Here's how the part is built. I have some questions about the finished solid (model axes, mm). A direction names the side the tool comes from. Coordinates: 2 decimals unless noted, no trailing zeros. Loops run counter-clockwise (first coordinate to the right, second up) from the corner with the lowest first, then second, coordinate; pieces in that order, holes last. Notation, with made-up numbers: (16.5, -27.75) -> (62.5, -27.75) arc R18 ccw to (62.5, -20.75) -> close; hole circle Ø4 at (24, 85.25). An arc over 180 degrees is marked (long way). Answer as a JSON object with one key per item and string values. Group by question number.
Q1. I want a section at A-A on y = 43. Write out the boundary of the cut face in (x, z).
Q2. I need wall thicknesses on line 1 (Z direction, x = 0, y = 80); line 2 (Z direction, x = 0, y = -6.5); line 3 (X direction, y = 84.5, z = -7.5). Which ranges of each line are inside material? Lowest first, please.
Q3. On a 3-axis mill with a long thin cutter (end or side, diameter ignored), from which of +Z, -Z, +X, -X, +Y, -Y can I reach the whole of each face in a straight line? I mean faces 1 (the cylindrical face through (-6.586, 73.801, -10.329)), 2 (the flat face through (7.3, 92.053, -10.1)), 3 (the cylindrical face through (2.285, -11.807, -3.584)), 4 (the flat face through (-14, 84, 0)), 5 (the flat face through (14, 84, 0)). Say none if no direction works.
Q4. I'm going to push flat-ended pins straight in: pin 1 (6 mm diameter, centred on x = -16.5, y = 47, fed in from +Z); pin 2 (12 mm diameter, centred on y = 40.5, z = -15.5, fed in from +X); pin 3 (7 mm diameter, centred on x = 0, z = 0, fed in from -Y); pin 4 (3 mm diameter, centred on x = -17, y = 8, fed in from +Z). Where does each tip first touch, or does it pass through?
```python
from build123d import *

# Parameters (mm, degrees)
CUT_EXTRUDE1_DEPTH      = 99.11063461
CUT_EXTRUDE1_DEPTH_BACK = 99.11063461
SKETCH2_W               = 1
SKETCH2_H               = 15
FILLET1_R               = 1
M27_TAPPED_HOLE1_D      = 24.5
M27_TAPPED_HOLE1_DEPTH  = 36
M27_TAPPED_HOLE1_TIP    = 7.360542583
M10_TAPPED_HOLE1_D      = 8.5
M10_TAPPED_HOLE1_DEPTH  = 20
M10_TAPPED_HOLE1_TIP    = 2.553657631


with BuildPart() as part:
    # Sketch1 → Revolve1 (revolve)
    with BuildSketch(Plane.XY):
        Polygon((0, 92.052683956), (0, -21.947316044), (-24, -21.947316044), (-24, -9.947316044), (-15, -9.947316044), (-15, 92.052683956), align=None)
    revolve(axis=Axis((0, 92.052683956, 0), (0, -1, 0)))

    # Sketch2 → Cut-Extrude1 (cut, two sides: drawn at the far end of the back side and taken through both)
    with BuildSketch(Plane.XY.offset(-CUT_EXTRUDE1_DEPTH_BACK)):
        with Locations((14.5, 84.552683956)):
            Rectangle(SKETCH2_W, SKETCH2_H)
        with Locations((-14.5, 84.552683956)):
            Rectangle(SKETCH2_W, SKETCH2_H)
    extrude(amount=CUT_EXTRUDE1_DEPTH + CUT_EXTRUDE1_DEPTH_BACK, mode=Mode.SUBTRACT)

    # Fillet1
    fillet1_edges = [part.edges().sort_by_distance(p)[0] for p in [
        (24, -9.947316044, 0),
        (24, -21.947316044, 0),
    ]]
    fillet(fillet1_edges, radius=FILLET1_R)

    # M27 Tapped Hole1
    with Locations(Plane(origin=(0, 92.052683956, 0), x_dir=(1, 0, 0), z_dir=(0, 1, 0))):
        with Locations((0, 0)):
            Hole(M27_TAPPED_HOLE1_D / 2, depth=M27_TAPPED_HOLE1_DEPTH)
            with Locations((0, 0, -(M27_TAPPED_HOLE1_DEPTH + M27_TAPPED_HOLE1_TIP / 2))):  # 118° drill point
                Cone(0, M27_TAPPED_HOLE1_D / 2, M27_TAPPED_HOLE1_TIP, mode=Mode.SUBTRACT)

    # M10 Tapped Hole1
    with Locations(Plane(origin=(0, -21.947316044, 0), x_dir=(-1, 0, 0), z_dir=(0, -1, 0))):
        with Locations((0, 0)):
            Hole(M10_TAPPED_HOLE1_D / 2, depth=M10_TAPPED_HOLE1_DEPTH)
            with Locations((0, 0, -(M10_TAPPED_HOLE1_DEPTH + M10_TAPPED_HOLE1_TIP / 2))):  # 118° drill point
                Cone(0, M10_TAPPED_HOLE1_D / 2, M10_TAPPED_HOLE1_TIP, mode=Mode.SUBTRACT)


solid = part.part
```
Result set:
{
 "1": {"outline": "circle Ø30 at (0, 0)"},
 "2": {"line 1": "z = -15 to -12.25, 12.25 to 15", "line 2": "z = -15 to -4.25, 4.25 to 15", "line 3": "x = -12.99 to -9.69, 9.69 to 12.99"},
 "3": {"face 1": "+Y", "face 2": "+Z, -Z, +X, -X, +Y", "face 3": "-Y", "face 4": "+Z, -Z, -X, +Y", "face 5": "+Z, -Z, +X, +Y"},
 "4": {"pin 1": "stops at z = 6.54", "pin 2": "stops at x = 11.61", "pin 3": "stops at y = -1.5", "pin 4": "passes through"}
}
